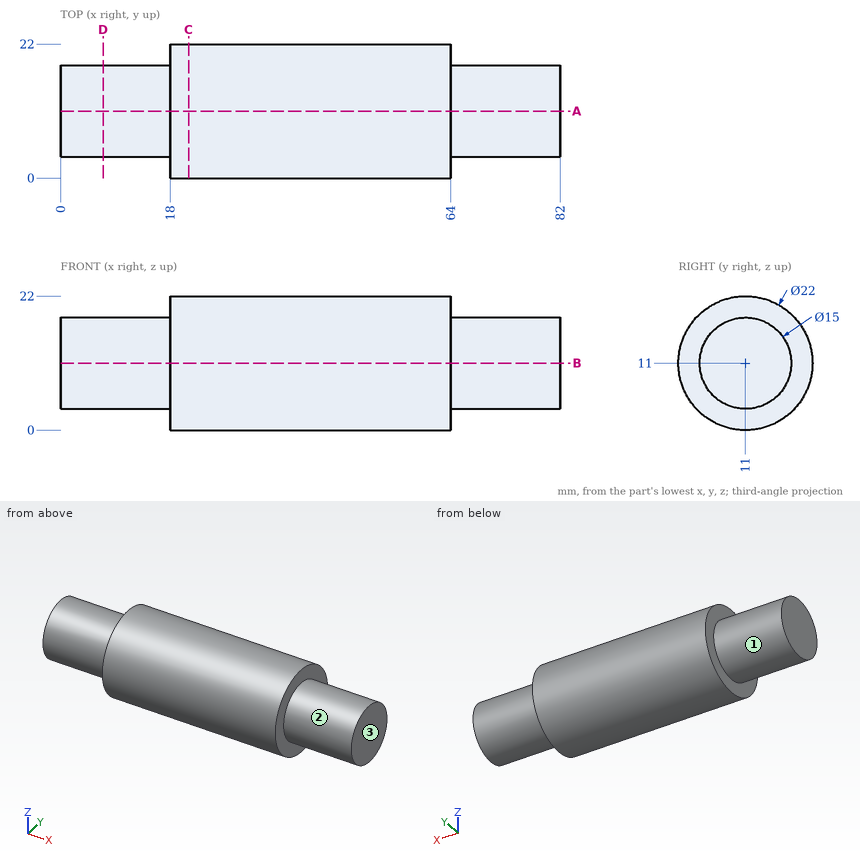
Can you work these out from the drawing? Everything is in mm from the part's minimum corner. A direction names the side the tool comes from. Round coordinates to 2 decimals unless told otherwise and drop trailing zeros. Loops run counter-clockwise (first coordinate to the right, second up) from the corner with the lowest first, then second, coordinate; pieces in that order, holes last. Notation, with made-up numbers: (14.25, 33.5) - (54.25, 33.5) arc R31 ccw to (54.25, 60.5) - close; hole circle Ø11 at (-28.75, 13.5). An arc over 180 degrees is marked (long way). Answer as CSV lines item,"result".
1. For pin 1 Ø3 at (x, y) = (15.5, 17.5) entering from +Z; pin 2 Ø1.5 at (x, y) = (9.5, 9.5) entering from -Z; pin 3 Ø6 at (x, z) = (24.5, 4.5) entering from +Y; pin 4 Ø11 at (y, z) = (7.5, 15.5) entering from -X, each with a flat end and sliding along its axis, tell me the tip position at first contact or that it passes through.
Filled in:
pin 1,"stops at z = 16.59"
pin 2,"stops at z = 3.54"
pin 3,"stops at y = 21.43"
pin 4,"stops at x = 0"
2. On a 3-axis mill with a long thin cutter (end or side, diameter ignored), from which of +Z, -Z, +X, -X, +Y, -Y can I reach the whole of each face in a straight line? I mean the marked faces 1, 2 and 3. Say none if no direction works.
Filled in:
face 1,"-X"
face 2,"+X"
face 3,"+Z, -Z, +X, +Y, -Y"
3. I want a section at C-C on x = 21. List the corners of the cut face in (y, z) for me.
Filled in:
outline,"circle Ø22 at (11, 11)"
4. Please list where these lines run through material, in increasing order: line 1 along X through (y, z) = (3.25, 18.25); line 2 along Z through (x, y) = (21, 11.5); line 3 along Y through (x, z) = (50, 10.75). Write a range as [from, to].
Filled in:
line 1,"x = [18, 64]"
line 2,"z = [0.01, 21.99]"
line 3,"y = [0, 22]"
5. I want a section at D-D on x = 7. List the corners of the cut face in (y, z) for me.
Filled in:
outline,"circle Ø15 at (11, 11)"
6. I want a section at A-A on y = 11. List the corners of the cut face in (x, z) for me, then the cut area to 3 significant figures.
Filled in:
outline,"(0, 3.5) - (18, 3.5) - (18, 0) - (64, 0) - (64, 3.5) - (82, 3.5) - (82, 18.5) - (64, 18.5) - (64, 22) - (18, 22) - (18, 18.5) - (0, 18.5) - close"
area,"1,550 mm^2"
